Here's how the part is built. I have some questions about the finished solid (model axes, mm). Face numbers are marked on the shaded views. Coordinates: 2 decimals unless noted, no trailing zeros. Loops run counter-clockwise (first coordinate to the right, second up) from the corner with the lowest first, then second, coordinate; pieces in that order, holes last. Notation, with made-up numbers: (36.5, 71.5) -> (41.5, 71.5) arc R27 ccw to (41.5, 91.5) -> close; hole circle Ø10 at (-20.75, -40). An arc over 180 degrees is marked (long way). Answer as a JSON object with one key per item and string values. Group by question number.
Q1. I want a section at D-D on z = 1.75. Write out the boundary of the cut face in (x, y), then the cut area to 3 significant figures.
Q2. I need wall thicknesses on line 1 (Y direction, x = 4, z = 7.75); line 2 (Y direction, x = 16, z = 2.25); line 3 (Z direction, x = -18, y = 5.5). Which ranges of each line are inside material? Lowest first, please.
Q3. I want a section at A-A on y = 0. Count the separate pieces of the cut face and the enclosed holes in it, then the cut area to 3 significant figures.
Q4. I want a section at C-C on x = -16. Write out the boundary of the cut face in (y, z), then the cut area to 3 significant figures.
Q5. I'm going to push flat-ended pins straight in: pin 1 (6 mm diameter, centred on x = 8.5, y = 5.5, fed in from -Z); pin 2 (2.5 mm diameter, centred on x = -16, y = 0, fed in from +Z); pin 3 (5.5 mm diameter, centred on x = 24, y = 0, fed in from +Z). Where does each tip first touch, or does it pass through?
Q6. Thinking about a two-plate mould opening in Y: for the marked faces 1, 2, 3 and 4, which applies, released by +Y, released by -Y, zero draft, split by the parting line, or undercut?
Q7. I want a section at B-B on z = 8.25. Write out the boundary of the cut face in (x, y).
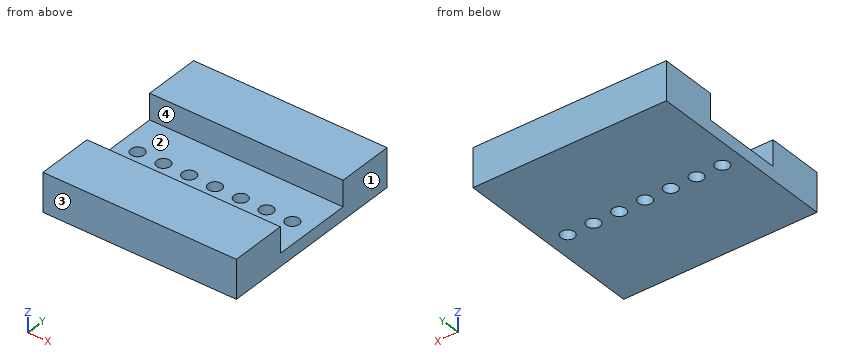
```python
from build123d import *

# Parameters (mm, degrees)
SKETCH_1_W             = 60
SKETCH_1_H             = 60
EXTRUDE_1_DEPTH        = 12
SKETCH_2_W             = 60
SKETCH_2_H             = 25
CUT_EXTRUDE_1_DEPTH    = 8
HOLE_WIZARD_M5_1_D     = 4.2
PATTERN_LINEAR_1_COUNT = 4
PATTERN_LINEAR_1_PITCH = 8
MIRROR_1_COPY_1_D      = 4.2
MIRROR_1_COPY_2_D      = 4.2
MIRROR_1_COPY_3_D      = 4.2
MIRROR_1_COPY_4_D      = 4.2


with BuildPart() as part:
    # 草图1 → 凸台-拉伸1 (new body)
    with BuildSketch(Plane.XY):
        Rectangle(SKETCH_1_W, SKETCH_1_H)
    extrude(amount=EXTRUDE_1_DEPTH)

    # 草图2 → 切除-拉伸1 (cut)
    with BuildSketch(Plane.XY.offset(12)):
        Rectangle(SKETCH_2_W, SKETCH_2_H)
    extrude(amount=-CUT_EXTRUDE_1_DEPTH, mode=Mode.SUBTRACT)

    # M5 螺纹孔1 (through all)
    with Locations(Plane.XY.offset(4)):
        with Locations((0, 0)):
            hole_wizard_m5_1 = Hole(HOLE_WIZARD_M5_1_D / 2)

    # 阵列(线性)1: M5 螺纹孔1 ×4
    with Locations(*[(-i * PATTERN_LINEAR_1_PITCH, 0, 0) for i in range(1, PATTERN_LINEAR_1_COUNT)]):
        add(hole_wizard_m5_1, mode=Mode.SUBTRACT)

    # 镜向1 copy 1 (through all)
    with Locations(Plane(origin=(8, 0, 4), x_dir=(-1, 0, 0), z_dir=(0, 0, 1))):
        with Locations((0, 0)):
            Hole(MIRROR_1_COPY_1_D / 2)

    # 镜向1 copy 2 (through all)
    with Locations(Plane(origin=(16, 0, 4), x_dir=(-1, 0, 0), z_dir=(0, 0, 1))):
        with Locations((0, 0)):
            Hole(MIRROR_1_COPY_2_D / 2)

    # 镜向1 copy 3 (through all)
    with Locations(Plane(origin=(24, 0, 4), x_dir=(-1, 0, 0), z_dir=(0, 0, 1))):
        with Locations((0, 0)):
            Hole(MIRROR_1_COPY_3_D / 2)

    # 镜向1 copy 4 (through all)
    with Locations(Plane(origin=(0, 0, 4), x_dir=(-1, 0, 0), z_dir=(0, 0, 1))):
        with Locations((0, 0)):
            Hole(MIRROR_1_COPY_4_D / 2)


solid = part.part
```
Result set:
{
 "1": {"outline": "(-30, -30) -> (30, -30) -> (30, 30) -> (-30, 30) -> close; hole circle Ø4.2 at (-24, 0); hole circle Ø4.2 at (-16, 0); hole circle Ø4.2 at (-8, 0); hole circle Ø4.2 at (0, 0); hole circle Ø4.2 at (8, 0); hole circle Ø4.2 at (16, 0); hole circle Ø4.2 at (24, 0)", "area": "3,500 mm²"},
 "2": {"line 1": "y = -30 to -12.5, 12.5 to 30", "line 2": "y = -30 to -2.1, 2.1 to 30", "line 3": "z = 0 to 4"},
 "3": {"separate pieces": "8", "enclosed holes": "0", "area": "122 mm²"},
 "4": {"outline": "(-30, 0) -> (-2.1, 0) -> (-2.1, 4) -> (-12.5, 4) -> (-12.5, 12) -> (-30, 12) -> close; (2.1, 0) -> (30, 0) -> (30, 12) -> (12.5, 12) -> (12.5, 4) -> (2.1, 4) -> close", "area": "503 mm²"},
 "5": {"pin 1": "stops at z = 0", "pin 2": "passes through", "pin 3": "stops at z = 4"},
 "6": {"face 1": "zero draft", "face 2": "undercut", "face 3": "released by -Y", "face 4": "undercut"},
 "7": {"outline": "(-30, -30) -> (30, -30) -> (30, -12.5) -> (-30, -12.5) -> close; (-30, 12.5) -> (30, 12.5) -> (30, 30) -> (-30, 30) -> close"}
}
